from build123d import *

# Parameters (mm, degrees)
BOSS_EXTRUDE1_DEPTH                                  = 15
M5_TAPPED_HOLE1_D                                    = 4.2
M5_TAPPED_HOLE1_DEPTH                                = 12.4
M5_TAPPED_HOLE1_CSINK_D                              = 5.05
M5_TAPPED_HOLE1_CSINK_ANGLE                          = 90
M5_TAPPED_HOLE1_TIP                                  = 1.2618073
CBORE_FOR_M8_HEXAGON_SOCKET_HEAD_CAP_SCR_D           = 9
CBORE_FOR_M8_HEXAGON_SOCKET_HEAD_CAP_SCR_CBORE_D     = 15
CBORE_FOR_M8_HEXAGON_SOCKET_HEAD_CAP_SCR_CBORE_DEPTH = 9
CBORE_FOR_M8_HEXAGON_SOCKET_HEAD_CAP_2_D             = 9
CBORE_FOR_M8_HEXAGON_SOCKET_HEAD_CAP_2_CBORE_D       = 15
CBORE_FOR_M8_HEXAGON_SOCKET_HEAD_CAP_2_CBORE_DEPTH   = 9
F_6_0MM_BLIND_HOLE_1_D                               = 6
FILLET1_R                                            = 5
CHAMFER1_SIZE                                        = 3


with BuildPart() as part:
    # Sketch1 → Boss-Extrude1 (new body)
    with BuildSketch(Plane(origin=(0, 0, 0), x_dir=(0, 0, -1), z_dir=(1, 0, 0))):
        Polygon((40, 0), (-40, 0), (-40, 80), (-25, 80), (-25, 180), (25, 180), (25, 80), (40, 80), align=None)
    extrude(amount=BOSS_EXTRUDE1_DEPTH)

    # M5 Tapped Hole1
    with Locations(Plane(origin=(15, 0, 0), x_dir=(0, 0, -1), z_dir=(1, 0, 0))):
        with Locations((31.5, 29), (-31.5, 29)):
            CounterSinkHole(M5_TAPPED_HOLE1_D / 2, M5_TAPPED_HOLE1_CSINK_D / 2, depth=M5_TAPPED_HOLE1_DEPTH, counter_sink_angle=M5_TAPPED_HOLE1_CSINK_ANGLE)
            with Locations((0, 0, -(M5_TAPPED_HOLE1_DEPTH + M5_TAPPED_HOLE1_TIP / 2))):  # 118° drill point
                Cone(0, M5_TAPPED_HOLE1_D / 2, M5_TAPPED_HOLE1_TIP, mode=Mode.SUBTRACT)

    # CBORE for M8 Hexagon socket head cap scr (through all)
    with Locations(Plane(origin=(15, 0, 0), x_dir=(0, 0, -1), z_dir=(1, 0, 0))):
        with Locations((0, 160), (0, 120)):
            CounterBoreHole(CBORE_FOR_M8_HEXAGON_SOCKET_HEAD_CAP_SCR_D / 2, CBORE_FOR_M8_HEXAGON_SOCKET_HEAD_CAP_SCR_CBORE_D / 2, CBORE_FOR_M8_HEXAGON_SOCKET_HEAD_CAP_SCR_CBORE_DEPTH)

    # CBORE for M8 Hexagon socket head cap 2 (through all)
    with Locations(Plane(origin=(15, 0, 0), x_dir=(0, 0, -1), z_dir=(1, 0, 0))):
        with Locations((-20, 15), (20, 15)):
            CounterBoreHole(CBORE_FOR_M8_HEXAGON_SOCKET_HEAD_CAP_2_D / 2, CBORE_FOR_M8_HEXAGON_SOCKET_HEAD_CAP_2_CBORE_D / 2, CBORE_FOR_M8_HEXAGON_SOCKET_HEAD_CAP_2_CBORE_DEPTH)

    # Ø6.0mm blind hole 1 (through all)
    with Locations(Plane(origin=(15, 0, 0), x_dir=(0, 0, -1), z_dir=(1, 0, 0))):
        with Locations((-20, 40), (20, 40)):
            Hole(F_6_0MM_BLIND_HOLE_1_D / 2)

    # Fillet1
    fillet1_edges = [part.edges().sort_by_distance(p)[0] for p in [
        (7.5, 80, 25),
        (7.5, 80, -25),
    ]]
    fillet(fillet1_edges, radius=FILLET1_R)

    # Chamfer1
    chamfer1_edges = [part.edges().sort_by_distance(p)[0] for p in [
        (7.5, 180, 25),
        (7.5, 180, -25),
        (7.5, 80, -40),
        (7.5, 0, -40),
        (7.5, 0, 40),
        (7.5, 80, 40),
    ]]
    chamfer(chamfer1_edges, length=CHAMFER1_SIZE)


solid = part.part
Source: CAD feature listing. Evaluate the final solid. Frame: model axes, mm. A direction names the side the tool comes from. Give positions to 0.01 mm unless a question says otherwise; leave off trailing zeros. Write each loop counter-clockwise with the first axis right and the second up, starting at its lowest first coordinate (ties: lowest second). Pieces come first, ordered by that corner, then holes. Notation, with made-up numbers: M 50,-7 L 69,-7 A27 cw 69,18 Z; hole C 24,26.5 d3. An arc over 180 degrees is marked long. Answer as a JSON object with one key per item and string values.
Q1. Cut plane A-A, the plane x = 11. Count the separate pieces of the cut face and the enclosed holes in it, then the cut area to 3 significant figures.
Geometry check:
{"separate pieces": "1", "enclosed holes": "8", "area": "10,600 mm^2"}
Q2. Cut plane B-B, the plane z = -20. Return the cut outline in (x, y).
Geometry check:
{"outline": "M 0,0 L 15,0 L 15,7.5 L 6,7.5 L 6,10.5 L 0,10.5 Z; M 0,19.5 L 6,19.5 L 6,22.5 L 15,22.5 L 15,37 L 0,37 Z; M 0,43 L 15,43 L 15,180 L 0,180 Z"}
Q3. Access query for faces 5 (the face through (6, 10, 20)), 6 (the face through (2.96, 18.04, -23.32)), 7 (the face through (7, 80, 34)), 8 (the face through (7, 132, -25)). Directions: +Z, -Z, +X, -X, +Y, -Y. A direction counts if a zero-diameter tool reaches every point of the face in a straight line with its end or side. Return the directions, or none.
Geometry check:
{"face 5": "+X", "face 6": "+X, -X", "face 7": "+Z, +X, -X, +Y", "face 8": "-Z, +X, -X, +Y"}
Q4. Mould query, pull axis Z, two halves, no side actions, for faces 1 (the face through (7, 78, -39)), 2 (the face through (6, 115, 0)), 3 (the face through (7, 130, 25)), 4 (the face through (7, 180, 0)). Classes: +Z half, -Z half, draft (parallel to the pull), parting line (faces both ways), or undercut.
Geometry check:
{"face 1": "-Z half", "face 2": "undercut", "face 3": "+Z half", "face 4": "draft"}
Q5. Contact query for flat-ended pins moving along their axis: P1, Ø7, axis at y = 160, z = 0, coming from the -X side (3 decimals); P2, Ø4, axis at y = 29, z = 31.5, coming from the +X side; P3, Ø4.5, axis at y = 18, z = 22, coming from the +X side; P4, Ø6, axis at x = 2.5, y = 80.5, coming from the -Z side. Output: stop coordinate, or through.
Geometry check:
{"P1": "passes through", "P2": "stops at x = 2.54", "P3": "stops at x = 6", "P4": "stops at z = -39.5"}
Q6. Ray query, line 1 along Y through (x, z) = (10.25, 0); line 2 along Y through (x, z) = (5.5, 20); line 3 along Z through (x, y) = (13, 14). Return the intervals inside material, ascending.
Geometry check:
{"line 1": "y = 0 to 112.5, 127.5 to 152.5, 167.5 to 180", "line 2": "y = 0 to 10.5, 19.5 to 37, 43 to 180", "line 3": "z = -40 to -27.43, -12.57 to 12.57, 27.43 to 40"}
Q7. Cut plane C-C, the plane y = 120. Return the cut outline in (x, z).
Geometry check:
{"outline": "M 0,-25 L 15,-25 L 15,-7.5 L 6,-7.5 L 6,-4.5 L 0,-4.5 Z; M 0,4.5 L 6,4.5 L 6,7.5 L 15,7.5 L 15,25 L 0,25 Z"}
Q8. Cut plane D-D, the plane y = 40. Return the cut outline in (x, z).
Geometry check:
{"outline": "M 0,-40 L 15,-40 L 15,-23 L 0,-23 Z; M 0,-17 L 15,-17 L 15,17 L 0,17 Z; M 0,23 L 15,23 L 15,40 L 0,40 Z"}
